For this review, take the finished solid that the model builds, in its own axes (mm). Face numbers are marked on the shaded views. A direction names the side the tool comes from. Give positions to 0.01 mm unless a question says otherwise; leave off trailing zeros. Loops run counter-clockwise (first coordinate to the right, second up) from the corner with the lowest first, then second, coordinate; pieces in that order, holes last. Notation, with made-up numbers: M -19.5,47.5 L 17.5,47.5 A7 cw 17.5,51.5 Z; hole C 53.25,-12 d9. An arc over 180 degrees is marked long. Use CSV: the item, a comma, the result in double quotes. Start each with the question number.
1. Take a section at B-B, the plane y = -10.5. Write out the cut boundary in (x, z).
2. Take a section at A-A, the plane z = -130. Write out the cut boundary in (x, y).
3. To check wall thickness, follow line 1 (Z direction, x = -23, y = 19); line 2 (X direction, y = 3, z = 163); line 3 (Y direction, x = -34.5, z = -91.5). State the ranges of each line that lie inside material, in increasing order. Write a range as [from, to].
4. Take a section at C-C, the plane x = -17. Write out the cut boundary in (y, z).
5. Tool access review of the marked faces 1 and 2: name each direction out of +Z, -Z, +X, -X, +Y, -Y from which nothing blocks a thin tool from reaching the whole face with its end or side.
6. Insertion check: P1, Ø11.5, axis at x = -14.5, z = -44.5, coming from the -Y side; P2, Ø2, axis at y = -1, z = 101.5, coming from the -X side. Each pin has a flat end and moves straight along its axis. Give the tip position at first contact, or say it passes through.
from build123d import *

# Parameters (mm, degrees)
SKETCH_1_W          = 420
SKETCH_1_H          = 40
EXTRUDE_1_DEPTH     = 1.5
SKETCH_2_W          = 420
SKETCH_2_H          = 1.5
EXTRUDE_2_DEPTH     = 40
FILLET_1_R          = 3
SKETCH_3_R          = 2.25
CUT_EXTRUDE_1_DEPTH = 10
SKETCH_6_R          = 2.25
CUT_EXTRUDE_2_DEPTH = 10
CUT_EXTRUDE_3_DEPTH = 218.214755484
CUT_EXTRUDE_4_DEPTH = 218.214755484


with BuildPart() as part:
    # 草图1 → 凸台-拉伸1 (new body)
    with BuildSketch(Plane(origin=(0, 0, 0), x_dir=(0, 0, -1), z_dir=(1, 0, 0))):
        Rectangle(SKETCH_1_W, SKETCH_1_H)
    extrude(amount=EXTRUDE_1_DEPTH)

    # 草图2 → 凸台-拉伸2 (add)
    with BuildSketch(Plane(origin=(1.5, 0, 0), x_dir=(0, 0, -1), z_dir=(1, 0, 0))):
        with Locations((0, 19.25)):
            Rectangle(SKETCH_2_W, SKETCH_2_H)
    extrude(amount=-EXTRUDE_2_DEPTH)

    # 圆角1
    fillet_1_edges = [part.edges().sort_by_distance(p)[0] for p in [
        (-38.5, 19.25, 210),
        (-38.5, 19.25, -210),
        (0.75, -20, -210),
        (0.75, -20, 210),
    ]]
    fillet(fillet_1_edges, radius=FILLET_1_R)

    # 草图3 → 切除-拉伸1 (cut)
    with BuildSketch(Plane(origin=(0, 20, 0), x_dir=(1, 0, 0), z_dir=(0, 1, 0))):
        with Locations(Location((-23.5, -95, 0), (0, 0, 270))):
            Circle(SKETCH_3_R)
        with Locations(Location((-23.5, 95, 0), (0, 0, 90))):
            Circle(SKETCH_3_R)
    extrude(amount=-CUT_EXTRUDE_1_DEPTH, mode=Mode.SUBTRACT)

    # 草图6 → 切除-拉伸2 (cut)
    with BuildSketch(Plane.XZ.offset(-18.5)):
        with Locations(Location((-23.5, -155, 0), (0, 0, 270))):
            Circle(SKETCH_6_R)
        with Locations(Location((-23.5, 155, 0), (0, 0, 270))):
            Circle(SKETCH_6_R)
    extrude(amount=-CUT_EXTRUDE_2_DEPTH, mode=Mode.SUBTRACT)

    # 草图7 → 切除-拉伸3 (cut, through all)
    with BuildSketch(Plane(origin=(0, 20, 0), x_dir=(1, 0, 0), z_dir=(0, 1, 0))):
        with BuildLine():
            Line((-10, -97.5), (-5, -97.5))
            ThreePointArc((-5, -97.5), (-2.5, -100), (-5, -102.5))
            Line((-5, -102.5), (-10, -102.5))
            ThreePointArc((-10, -102.5), (-12.5, -100), (-10, -97.5))
        make_face()
        with BuildLine():
            Line((-5, 47.5), (-10, 47.5))
            ThreePointArc((-10, 47.5), (-12.5, 50), (-10, 52.5))
            Line((-10, 52.5), (-5, 52.5))
            ThreePointArc((-5, 52.5), (-2.5, 50), (-5, 47.5))
        make_face()
    extrude(amount=-CUT_EXTRUDE_3_DEPTH, mode=Mode.SUBTRACT)

    # 草图9 → 切除-拉伸4 (cut, through all)
    with BuildSketch(Plane(origin=(0, 20, 0), x_dir=(1, 0, 0), z_dir=(0, 1, 0))):
        with BuildLine():
            Line((-5, -52.5), (-10, -52.5))
            ThreePointArc((-10, -52.5), (-12.5, -50), (-10, -47.5))
            Line((-10, -47.5), (-5, -47.5))
            ThreePointArc((-5, -47.5), (-2.5, -50), (-5, -52.5))
        make_face()
        with BuildLine():
            Line((-5, 97.5), (-10, 97.5))
            ThreePointArc((-10, 97.5), (-12.5, 100), (-10, 102.5))
            Line((-10, 102.5), (-5, 102.5))
            ThreePointArc((-5, 102.5), (-2.5, 100), (-5, 97.5))
        make_face()
    extrude(amount=-CUT_EXTRUDE_4_DEPTH, mode=Mode.SUBTRACT)


solid = part.part
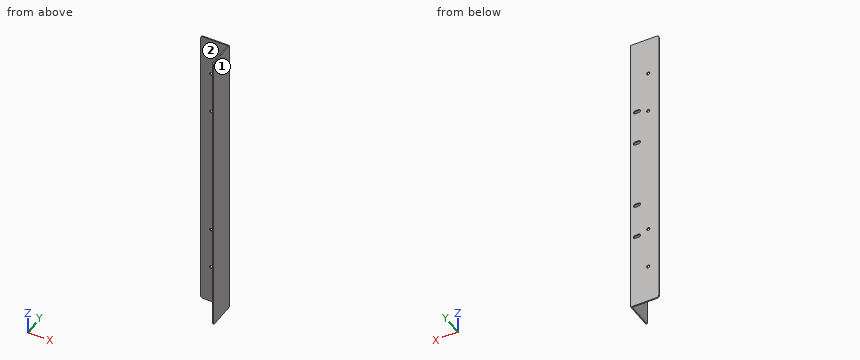
Result set:
1,outline,"M 0,-210 L 1.5,-210 L 1.5,210 L 0,210 Z"
2,outline,"M -38.5,18.5 L 0,18.5 L 0,-20 L 1.5,-20 L 1.5,20 L -38.5,20 Z"
3,line 1,"[-210, -157.19], [-152.81, -97.19], [-92.81, 92.81], [97.19, 152.81], [157.19, 210]"
3,line 2,"[0, 1.5]"
3,line 3,"[18.5, 20]"
4,outline,"M 18.5,-210 L 20,-210 L 20,210 L 18.5,210 Z"
5,face 1,"+Z, -Z, +X, +Y, -Y"
5,face 2,"+Z, -Z, -X, -Y"
6,P1,"y = 18.5"
6,P2,"x = 0"
